For this review, use the dimensioned drawing (mm, ordinates from the lowest corner) and the shaded views. A direction names the side the tool comes from. Round coordinates to 2 decimals unless told otherwise and drop trailing zeros. Loops run counter-clockwise (first coordinate to the right, second up) from the corner with the lowest first, then second, coordinate; pieces in that order, holes last. Notation, with made-up numbers: (29, 1.25) - (33, 1.25) arc R25 cw to (33, 16.25) - close; hole circle Ø8 at (83.5, 20). An arc over 180 degrees is marked (long way). Return JSON: item names as keys, results as strings. Group by question number.
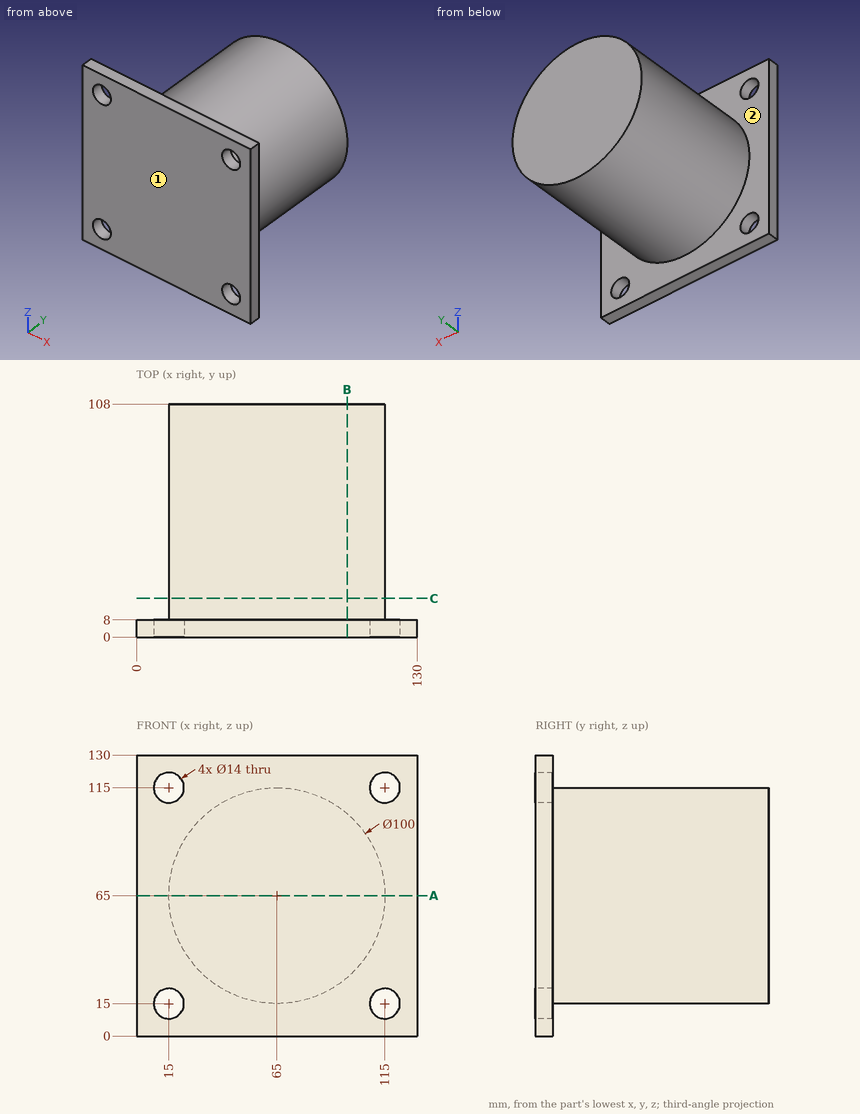
Q1. Add section C-C, the plane y = 18. State the section outline as (x, z) points.
Q2. Add section B-B, the plane x = 97.5. State the section outline as (y, z) points.
Q3. Tool access review of the marked faces 1 and 2: name each direction out of +Z, -Z, +X, -X, +Y, -Y from which nothing blocks a thin tool from reaching the whole face with its end or side.
Q4. Insertion check: pin 1 Ø10 at (x, z) = (37, 91.5) entering from -Y; pin 2 Ø18 at (x, z) = (15, 115) entering from +Y; pin 3 Ø3 at (x, y) = (96.5, 31) entering from +Z; pin 4 Ø1 at (y, z) = (85.5, 57.5) entering from -X. Each pin has a flat end and moves straight along its axis. Give the tip position at first contact, or say it passes through.
Q5. For line 1 (X direction, y = 6, z = 15); line 2 (Y direction, x = 25, z = 8.5), list the stretches that pass through material, from the lowest coordinate up.
Q6. Add section A-A, the plane z = 65. State the section outline as (x, y) points, plus the area to 3 significant figures.
Evaluation:
{
 "1": {"outline": "circle Ø100 at (65, 65)"},
 "2": {"outline": "(0, 0) - (8, 0) - (8, 27) - (108, 27) - (108, 103) - (8, 103) - (8, 130) - (0, 130) - close"},
 "3": {"face 1": "+Z, -Z, +X, -X, -Y", "face 2": "+Y"},
 "4": {"pin 1": "y = 0", "pin 2": "y = 8", "pin 3": "z = 105", "pin 4": "x = 15.49"},
 "5": {"line 1": "0 to 8, 22 to 108, 122 to 130", "line 2": "0 to 8"},
 "6": {"outline": "(0, 0) - (130, 0) - (130, 8) - (115, 8) - (115, 108) - (15, 108) - (15, 8) - (0, 8) - close", "area": "11,000 mm²"}
}
